from build123d import *

# Parameters (mm, degrees)
SKETCH_1_W      = 80
SKETCH_1_H      = 60
EXTRUDE_1_DEPTH = 1264
FILLET_1_R      = 5
SHELL_1_T       = -3


with BuildPart() as part:
    # 草图1 → 凸台-拉伸1 (new body)
    with BuildSketch(Plane.XY):
        Rectangle(SKETCH_1_W, SKETCH_1_H)
    extrude(amount=EXTRUDE_1_DEPTH)

    # 圆角1
    fillet_1_edges = [part.edges().sort_by_distance(p)[0] for p in [
        (-40, 30, 632),
        (40, 30, 632),
        (40, -30, 632),
        (-40, -30, 632),
    ]]
    fillet(fillet_1_edges, radius=FILLET_1_R)

    # 抽壳1
    shell_1_openings = [part.faces().sort_by_distance(p)[0] for p in [
        (0, 0, 1264),
        (0, 0, 0),
    ]]
    offset(amount=SHELL_1_T, openings=shell_1_openings, kind=Kind.INTERSECTION)


solid = part.part
Work out the finished part from the listing and answer in its coordinate system (mm). A direction names the side the tool comes from. Give positions to 0.01 mm unless a question says otherwise; leave off trailing zeros. Loops run counter-clockwise (first coordinate to the right, second up) from the corner with the lowest first, then second, coordinate; pieces in that order, holes last. Notation, with made-up numbers: (77.25, -18) - (111.25, -18) arc R30 cw to (111.25, 21) - close; hole circle Ø11 at (-26.5, 38). An arc over 180 degrees is marked (long way). Answer in a Markdown table with one row per item.
(1) Consider L1, parallel to Y at x = 1, z = 402.5; L2, parallel to X at y = 24.5, z = 314. Determine where each line is inside the solid, lowest interval first. Write a range as [from, to].
Results list:
| item | result |
|---|---|
| L1 | y = [-30, -27], [27, 30] |
| L2 | x = [-40, -37], [37, 40] |
(2) Section B-B (y = 8) is taken. Give the vertices of the cut face in (x, z).
Results list:
| item | result |
|---|---|
| outline | (-40, 0) - (-37, 0) - (-37, 1264) - (-40, 1264) - close; (37, 0) - (40, 0) - (40, 1264) - (37, 1264) - close |
(3) For a pull along Y with two mould halves and no side action, classify faces 1 (the face through (-37, 0, 623)), 2 (the face through (0, 30, 623)), 3 (the face through (-40, 0, 623)) as pulls with the +Y half, pulls with the -Y half, needs draft (parallel to the pull), parting line crosses it, or undercut.
Results list:
| item | result |
|---|---|
| face 1 | undercut |
| face 2 | pulls with the +Y half |
| face 3 | needs draft |
(4) Section C-C (z = 1167.5) is taken. Give the vertices of the cut face in (x, y).
Results list:
| item | result |
|---|---|
| outline | (-40, -25) arc R5 ccw to (-35, -30) - (35, -30) arc R5 ccw to (40, -25) - (40, 25) arc R5 ccw to (35, 30) - (-35, 30) arc R5 ccw to (-40, 25) - close; hole (-37, -25) arc R2 ccw to (-35, -27) - (35, -27) arc R2 ccw to (37, -25) - (37, 25) arc R2 ccw to (35, 27) - (-35, 27) arc R2 ccw to (-37, 25) - close |
(5) Section A-A (x = -5.5) is taken. Give the vertices of the cut face in (y, z), and give its area (3 significant figures).
Results list:
| item | result |
|---|---|
| outline | (-30, 0) - (-27, 0) - (-27, 1264) - (-30, 1264) - close; (27, 0) - (30, 0) - (30, 1264) - (27, 1264) - close |
| area | 7,580 mm² |
(6) A tool of negligible diameter and unlimited length cuts with its end or side. For faces 4 (the face through (0, -27, 623)), 5 (the face through (0, -30, 623)), from which of +Z, -Z, +X, -X, +Y, -Y can it reach the whole face along a straight path? Write none if from no direction.
Results list:
| item | result |
|---|---|
| face 4 | +Z, -Z |
| face 5 | +Z, -Z, +X, -X, -Y |
